```python
from build123d import *

# Parameters (mm, degrees)
SKETCH1_W             = 60
SKETCH1_H             = 60
BOSS_EXTRUDE1_DEPTH   = 10
FILLET1_R             = 5
M6_TAPPED_HOLE1_D     = 5
M6_TAPPED_HOLE1_DEPTH = 15
M6_TAPPED_HOLE1_TIP   = 1.502151548
SKETCH8_R             = 2.1
CUT_EXTRUDE1_DEPTH    = 51.336896077
SKETCH9_R             = 4
CUT_EXTRUDE2_DEPTH    = 5
M4_TAPPED_HOLE1_D     = 3.3
M4_TAPPED_HOLE2_D     = 3.3
SKETCH15_R            = 4
CUT_EXTRUDE3_DEPTH    = 5
SKETCH16_R            = 2.1
CUT_EXTRUDE4_DEPTH    = 51.336896077


with BuildPart() as part:
    # Sketch1 → Boss-Extrude1 (new body)
    with BuildSketch(Plane.XY):
        with Locations((9.163798419, 0)):
            Rectangle(SKETCH1_W, SKETCH1_H)
    extrude(amount=BOSS_EXTRUDE1_DEPTH)

    # Fillet1
    fillet1_edges = [part.edges().sort_by_distance(p)[0] for p in [
        (-20.836201581, 30, 5),
        (39.163798419, 30, 5),
        (39.163798419, -30, 5),
        (-20.836201581, -30, 5),
    ]]
    fillet(fillet1_edges, radius=FILLET1_R)

    # M6 Tapped Hole1
    with Locations(Plane.XY.offset(10)):
        with Locations((9.163798419, -21.25), (30.814433514, 16.25), (-12.486836675, 16.25)):
            Hole(M6_TAPPED_HOLE1_D / 2, depth=M6_TAPPED_HOLE1_DEPTH)
            with Locations((0, 0, -(M6_TAPPED_HOLE1_DEPTH + M6_TAPPED_HOLE1_TIP / 2))):  # 118° drill point
                Cone(0, M6_TAPPED_HOLE1_D / 2, M6_TAPPED_HOLE1_TIP, mode=Mode.SUBTRACT)

    # Sketch8 → Cut-Extrude1 (cut, through all)
    with BuildSketch(Plane.XY.offset(10)):
        with Locations((9.163798419, 25)):
            Circle(SKETCH8_R)
        with Locations((34.163798419, 0)):
            Circle(SKETCH8_R)
        with Locations((-15.836201581, 0)):
            Circle(SKETCH8_R)
    extrude(amount=-CUT_EXTRUDE1_DEPTH, mode=Mode.SUBTRACT)

    # Sketch9 → Cut-Extrude2 (cut)
    with BuildSketch(Plane.XY.offset(10)):
        with Locations((-15.836201581, 0)):
            Circle(SKETCH9_R)
        with Locations((9.163798419, 25)):
            Circle(SKETCH9_R)
        with Locations((34.163798419, 0)):
            Circle(SKETCH9_R)
    extrude(amount=-CUT_EXTRUDE2_DEPTH, mode=Mode.SUBTRACT)

    # M4 Tapped Hole1 (through all)
    with Locations(Plane.XY.offset(10)):
        with Locations((-15.836201581, -25), (34.163798419, -25), (34.163798419, 25), (-15.836201581, 25)):
            Hole(M4_TAPPED_HOLE1_D / 2)

    # M4 Tapped Hole2 (through all)
    with Locations(Plane.XY.offset(10)):
        with Locations((9.163798419, 0)):
            Hole(M4_TAPPED_HOLE2_D / 2)

    # Sketch15 → Cut-Extrude3 (cut)
    with BuildSketch(Plane.XY.offset(10)):
        with Locations((9.163798419, 0)):
            Circle(SKETCH15_R)
    extrude(amount=-CUT_EXTRUDE3_DEPTH, mode=Mode.SUBTRACT)

    # Sketch16 → Cut-Extrude4 (cut, through all)
    with BuildSketch(Plane.XY.offset(10)):
        with Locations((9.163798419, 0)):
            Circle(SKETCH16_R)
    extrude(amount=-CUT_EXTRUDE4_DEPTH, mode=Mode.SUBTRACT)


solid = part.part
```
The model under review builds one solid part; all positions refer to its coordinate system, in mm. A direction names the side the tool comes from. Round coordinates to 2 decimals unless told otherwise and drop trailing zeros. Loops run counter-clockwise (first coordinate to the right, second up) from the corner with the lowest first, then second, coordinate; pieces in that order, holes last. Notation, with made-up numbers: M -23.75,60.5 L -9.75,60.5 A7 cw -9.75,72.5 Z; hole C -14,-0.75 d11. An arc over 180 degrees is marked long. Write item = value, one per line.
Item 1: The part is to be moulded in two halves that separate along X. For faces 1 (the flat face through (39.164, 0, 5)), 2 (the flat face through (9, -30, 5)), 3 (the cylindrical face through (-19.41, -28.496, 5.07)), 4 (the flat face through (11, -2, 5)), say which applies: released by +X, released by -X, zero draft, split by the parting line, or undercut.
Return value:
face_1 = released by +X
face_2 = zero draft
face_3 = released by -X
face_4 = undercut
Item 2: Take a section at C-C on z = 2.75. State how many separate pieces and enclosed holes the cut face has, then the cut area to 3 significant figures.
Return value:
separate_pieces = 1
enclosed_holes = 11
area = 3,430 mm2
Item 3: Take a section at B-B on y = 16.25. Write out the cut boundary in (x, z), then the cut area to 3 significant figures.
Return value:
outline = M -20.84,0 L -14.99,0 L -14.99,10 L -20.84,10 Z; M -9.99,0 L 28.31,0 L 28.31,10 L -9.99,10 Z; M 33.31,0 L 39.16,0 L 39.16,10 L 33.31,10 Z
area = 500 mm2
Item 4: For line 1 (X direction, y = 1, z = 3.5); line 2 (Y direction, x = 7.5, z = 0.5); line 3 (Y direction, x = 11, z = 5.5), list the stretches that pass through material, from the lowest coordinate up. Write a range as [from, to].
Return value:
line_1 = [-20.84, -17.68], [-13.99, 7.32], [11.01, 32.32], [36.01, 39.16]
line_2 = [-30, -23.12], [-19.38, -1.28], [1.28, 23.72], [26.28, 30]
line_3 = [-30, -22.95], [-19.55, -3.55], [3.55, 21.45], [28.55, 30]
Item 5: Take a section at A-A on y = 0. Write out the cut boundary in (x, z).
Return value:
outline = M -20.84,0 L -17.94,0 L -17.94,5 L -19.84,5 L -19.84,10 L -20.84,10 Z; M -13.74,0 L 7.06,0 L 7.06,5 L 5.16,5 L 5.16,10 L -11.84,10 L -11.84,5 L -13.74,5 Z; M 11.26,0 L 32.06,0 L 32.06,5 L 30.16,5 L 30.16,10 L 13.16,10 L 13.16,5 L 11.26,5 Z; M 36.26,0 L 39.16,0 L 39.16,10 L 38.16,10 L 38.16,5 L 36.26,5 Z
Item 6: Take a section at D-D on y = -21.25. Write out the cut boundary in (x, z), then the cut area to 3 significant figures.
Return value:
outline = M -20.84,0 L 6.66,0 L 6.66,10 L -20.84,10 Z; M 11.66,0 L 39.16,0 L 39.16,10 L 11.66,10 Z
area = 550 mm2
Item 7: Insertion check: P1, Ø4, axis at x = 7.5, y = 25.5, coming from the +Z side. The pin has a flat end and moves straight along its axis. Give the tip position at first contact, or say it passes through.
Return value:
P1 = 5
Item 8: Machinability: for faces 5 (the flat face through (11, 23, 5)), 6 (the cylindrical face through (-15.621, -23.364, 4.93)), which of the approach directions +Z, -Z, +X, -X, +Y, -Y give a long, thin tool a straight path to every point of the face, cutting with its end or side? Answer none if there is none.
Return value:
face_5 = +Z
face_6 = +Z, -Z
